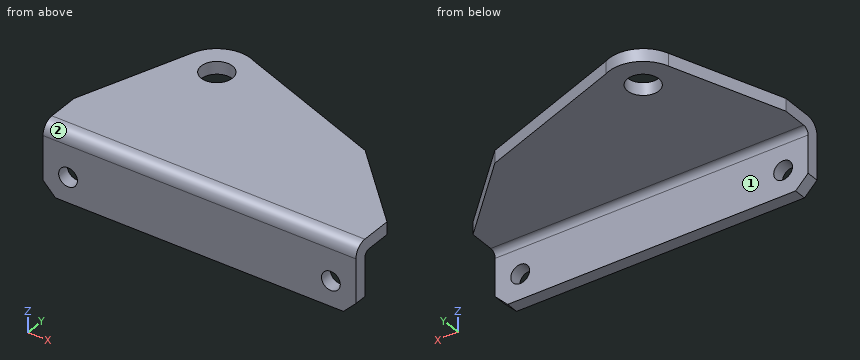
from build123d import *

# Parameters (mm, degrees)
SKETCH1_W           = 250
SKETCH1_H           = 181
BOSS_EXTRUDE1_DEPTH = 10
SKETCH2_OUTSIDE_W   = 313.762
SKETCH2_OUTSIDE_H   = 244.762
CUT_EXTRUDE1_DEPTH  = 10
SKETCH3_R           = 12.5
CUT_EXTRUDE2_DEPTH  = 10
SKETCH4_W           = 250
SKETCH4_H           = 10
BOSS_EXTRUDE2_DEPTH = 45
FILLET1_R           = 10
FILLET2_R           = 5
SKETCH5_R           = 7.5
CUT_EXTRUDE3_DEPTH  = 45
CHAMFER1_SIZE       = 10


with BuildPart() as part:
    # Sketch1 → Boss-Extrude1 (new body)
    with BuildSketch(Plane.XY):
        Rectangle(SKETCH1_W, SKETCH1_H)
    extrude(amount=BOSS_EXTRUDE1_DEPTH)

    # Sketch2 outside → Cut-Extrude1 (cut)
    with BuildSketch(Plane.XY.offset(10)):
        Rectangle(SKETCH2_OUTSIDE_W, SKETCH2_OUTSIDE_H)
        with BuildLine():
            Line((-125, -55.5), (-93.159896838, 31.97996447))
            ThreePointArc((-93.159896838, 31.97996447), (-77.523014584, 48.907010136), (-54.496896373, 47.993313367))
            Line((-54.496896373, 47.993313367), (65, 4.5))
            Line((65, 4.5), (125, -55.5))
            Line((125, -55.5), (125, -90.5))
            Line((125, -90.5), (-125, -90.5))
            Line((-125, -90.5), (-125, -55.5))
        make_face(mode=Mode.SUBTRACT)
    extrude(amount=-CUT_EXTRUDE1_DEPTH, mode=Mode.SUBTRACT)

    # Sketch3 → Cut-Extrude2 (cut)
    with BuildSketch(Plane.XY.offset(10)):
        with Locations((-67, 23.5)):
            Circle(SKETCH3_R)
    extrude(amount=-CUT_EXTRUDE2_DEPTH, mode=Mode.SUBTRACT)

    # Sketch4 → Boss-Extrude2 (add)
    with BuildSketch(Plane(origin=(0, 0, 0), x_dir=(-1, 0, 0), z_dir=(0, 0, -1))):
        with Locations((0, -85.5)):
            Rectangle(SKETCH4_W, SKETCH4_H)
    extrude(amount=BOSS_EXTRUDE2_DEPTH)

    # Fillet1
    fillet1_edges = [part.edges().sort_by_distance(p)[0] for p in [
        (0, -90.5, 10),
    ]]
    fillet(fillet1_edges, radius=FILLET1_R)

    # Fillet2
    fillet2_edges = [part.edges().sort_by_distance(p)[0] for p in [
        (0, -80.5, 0),
    ]]
    fillet(fillet2_edges, radius=FILLET2_R)

    # Sketch5 → Cut-Extrude3 (cut)
    with BuildSketch(Plane.XZ.offset(90.5)):
        with Locations((-105, -25)):
            Circle(SKETCH5_R)
        with Locations((105, -25)):
            Circle(SKETCH5_R)
    extrude(amount=-CUT_EXTRUDE3_DEPTH, mode=Mode.SUBTRACT)

    # Chamfer1
    chamfer1_edges = [part.edges().sort_by_distance(p)[0] for p in [
        (125, -85.5, -45),
        (-125, -85.5, -45),
    ]]
    chamfer(chamfer1_edges, length=CHAMFER1_SIZE)


solid = part.part
The model under review builds one solid part; all positions refer to its coordinate system, in mm. Face numbers are marked on the shaded views. A direction names the side the tool comes from. Coordinates: 2 decimals unless noted, no trailing zeros. Write each loop counter-clockwise with the first axis right and the second up, starting at its lowest first coordinate (ties: lowest second). Pieces come first, ordered by that corner, then holes. Notation, with made-up numbers: (-22.75, -10.75) -> (-13.75, -10.75) arc R35 cw to (-13.75, 23.25) -> close; hole circle Ø4 at (9.25, 42). An arc over 180 degrees is marked (long way). Answer in a Markdown table with one row per item.
1. We need section B-B, the plane y = 17. State the section outline as (x, z) points, and give its area (3 significant figures).
Answers below:
| item | result |
|---|---|
| outline | (-98.61, 0) -> (-77.68, 0) -> (-77.68, 10) -> (-98.61, 10) -> close; (-56.32, 0) -> (30.66, 0) -> (30.66, 10) -> (-56.32, 10) -> close |
| area | 1,080 mm^2 |
2. We need section D-D, the plane x = 105. State the section outline as (y, z) points.
Answers below:
| item | result |
|---|---|
| outline | (-90.5, -45) -> (-80.5, -45) -> (-80.5, -32.5) -> (-90.5, -32.5) -> close; (-90.5, -17.5) -> (-80.5, -17.5) -> (-80.5, -5) arc R5 cw to (-75.5, 0) -> (-35.5, 0) -> (-35.5, 10) -> (-80.5, 10) arc R10 ccw to (-90.5, 0) -> close |
3. For the marked faces 1 and 2, list the 3-axis set-ups (+Z, -Z, +X, -X, +Y, -Y) from which the entire face can be reached by the end or side of a thin tool; tool diameter is ignored.
Answers below:
| item | result |
|---|---|
| face 1 | -Z, +X, -X, +Y |
| face 2 | +Z, +X, -X, -Y |
4. We need section C-C, the plane z = -25. State the section outline as (x, y) points, and give its area (3 significant figures).
Answers below:
| item | result |
|---|---|
| outline | (-125, -90.5) -> (-112.5, -90.5) -> (-112.5, -80.5) -> (-125, -80.5) -> close; (-97.5, -90.5) -> (97.5, -90.5) -> (97.5, -80.5) -> (-97.5, -80.5) -> close; (112.5, -90.5) -> (125, -90.5) -> (125, -80.5) -> (112.5, -80.5) -> close |
| area | 2,200 mm^2 |
5. Wall thickness on probe 1 along Z at (x, y) = (34, 7); probe 2 along Z at (x, y) = (105, -83); probe 3 along Y at (x, z) = (81, -14): over which ranges is each line inside the solid? List them lowest first. Write a range as [from, to].
Answers below:
| item | result |
|---|---|
| probe 1 | z = [0, 10] |
| probe 2 | z = [-45, -32.5], [-17.5, 9.68] |
| probe 3 | y = [-90.5, -80.5] |
6. Clearance check with flat-ended pins moving along their axes: pin 1 Ø19.5 at (x, z) = (105, -25) entering from +Y; pin 2 Ø10 at (y, z) = (-31.5, 1) entering from -X; pin 3 Ø10 at (x, y) = (-72.5, -55) entering from -Z. State where each tip first meets the part, or that it passes through.
Answers below:
| item | result |
|---|---|
| pin 1 | stops at y = -80.5 |
| pin 2 | stops at x = -118.08 |
| pin 3 | stops at z = 0 |
7. We need section A-A, the plane x = -67. State the section outline as (y, z) points, and give its area (3 significant figures).
Answers below:
| item | result |
|---|---|
| outline | (-90.5, -45) -> (-80.5, -45) -> (-80.5, -5) arc R5 cw to (-75.5, 0) -> (11, 0) -> (11, 10) -> (-80.5, 10) arc R10 ccw to (-90.5, 0) -> close; (36, 0) -> (51, 0) -> (51, 10) -> (36, 10) -> close |
| area | 1,600 mm^2 |
